Verification items for the finished model (mm, model axes). A direction names the side the tool comes from. Coordinates: 2 decimals unless noted, no trailing zeros. Write each loop counter-clockwise with the first axis right and the second up, starting at its lowest first coordinate (ties: lowest second). Pieces come first, ordered by that corner, then holes. Notation, with made-up numbers: (18.5, -36) -> (27.5, -36) arc R11 ccw to (27.5, -27) -> close; hole circle Ø10 at (73.25, -29.75). An arc over 180 degrees is marked (long way). Answer in a Markdown table with one row per item.
```python
from build123d import *

# Parameters (mm, degrees)
BARREL_PROFILE_SKETCH_R  = 115
BARREL_BODY_230_DEPTH    = 1100
EYE_PIN_HOLE_SKETCH_R    = 50.25
EYE_PIN_HOLE_100_5_DEPTH = 1100
EYE_FLATS_SKETCH_W       = 230
EYE_FLATS_SKETCH_H       = 365
EYE_FLATS_CUT_DEPTH      = 2200
EYE_START                = -117
EYE_BOSS_SKETCH_R        = 115
EYE_BOSS_SKETCH_R_2      = 50.25
EYE_BOSS_EXTRUDE_DEPTH   = 117
EDGE_FILLET_R10_R        = 10


with BuildPart() as part:
    # Barrel Profile Sketch → Barrel Body Ø230 (new, symmetric)
    with BuildSketch(Plane.XY):
        Circle(BARREL_PROFILE_SKETCH_R)
    extrude(amount=BARREL_BODY_230_DEPTH, both=True)

    # Eye Pin Hole Sketch → Eye Pin Hole Ø100.5 (cut, symmetric)
    with BuildSketch(Plane(origin=(0, 0, 0), x_dir=(1, 0, 0), z_dir=(0, 1, 0))):
        with Locations(Location((0, 955, 0), (0, 0, 270))):
            Circle(EYE_PIN_HOLE_SKETCH_R)
    extrude(amount=EYE_PIN_HOLE_100_5_DEPTH, both=True, mode=Mode.SUBTRACT)

    # Eye Flats Sketch → Eye Flats Cut (cut)
    with BuildSketch(Plane(origin=(0, 0, 0), x_dir=(1, 0, 0), z_dir=(0, 1, 0))):
        with Locations((0, 917.5)):
            Rectangle(EYE_FLATS_SKETCH_W, EYE_FLATS_SKETCH_H)
    extrude(amount=-EYE_FLATS_CUT_DEPTH, mode=Mode.SUBTRACT)

    # Eye Transition Sketch → Eye Transition Revolve Cut (revolve, cut)
    with BuildSketch(Plane.XZ):
        with BuildLine():
            Line((-115, -955), (-196.346531204, -955))
            Line((-196.346531204, -955), (-196.346531204, -1191.859792513))
            Line((-196.346531204, -1191.859792513), (0, -1191.859792513))
            Line((0, -1191.859792513), (0, -1070))
            ThreePointArc((0, -1070), (-81.317279836, -1036.317279836), (-115, -955))
        make_face()
    revolve(axis=Axis((0, 0, -1191.859792513), (0, 0, 1)), mode=Mode.SUBTRACT)

    # End Bore Sketch → End Bore Revolve Cut (revolve, cut)
    with BuildSketch(Plane(origin=(0, 0, 0), x_dir=(1, 0, 0), z_dir=(0, 1, 0))):
        Polygon((0, -1100), (61, -1100), (61, -1055.102870795), (81, -1055.102870795), (81, 685), (0, 685), align=None)
    revolve(axis=Axis((0, 0, 1100), (0, 0, -1)), mode=Mode.SUBTRACT)

    # Eye Boss Sketch → Eye Boss Extrude (add)
    with BuildSketch(Plane.XZ.offset(EYE_START)):
        with Locations(Location((0, -955, 0), (0, 0, 270))):
            Circle(EYE_BOSS_SKETCH_R)
        with Locations(Location((0, -955, 0), (0, 0, 90))):
            Circle(EYE_BOSS_SKETCH_R_2, mode=Mode.SUBTRACT)
    extrude(amount=EYE_BOSS_EXTRUDE_DEPTH)

    # Edge Fillet R10
    edge_fillet_r10_edges = [part.edges().sort_by_distance(p)[0] for p in [
        (-115, 0, 1100),
    ]]
    fillet(edge_fillet_r10_edges, radius=EDGE_FILLET_R10_R)


solid = part.part
```
1. Thickness scan on line 1 (Z direction, x = 0, y = 74); line 2 (X direction, y = 0, z = 629); line 3 (Z direction, x = 0, y = 106). Record the ranges inside material, lowest first. Write a range as from..to.
Geometry says:
| item | result |
|---|---|
| line 1 | -1070..-1005.25, -904.75..-685, 1055.1..1100 |
| line 2 | -115..-81, 81..115 |
| line 3 | -1070..-1005.25, -904.75..1099.95 |
2. Mould release check, pull along Z, two halves, no side actions. Record for faces 6 (the cylindrical face through (34.54, 59.32, -1064.69)), 7 (the cylindrical face through (-48.408, 37.118, 1077.237)), 8 (the cylindrical face through (43.545, -68.3, 172.871)): released by +Z, released by -Z, zero draft, split by the parting line, or undercut.
Geometry says:
| item | result |
|---|---|
| face 6 | split by the parting line |
| face 7 | zero draft |
| face 8 | undercut |
3. Section check C-C, the plane z = -796.5. Record the boundary of the cut face in (x, y).
Geometry says:
| item | result |
|---|---|
| outline | (-115, 0) -> (115, 0) arc R115 ccw to start |
4. Depth check by flat-ended pin: P1, Ø2, axis at x = -46, z = 268, coming from the -Y side; P2, Ø1, axis at y = -55.5, z = 714, coming from the -X side; P3, Ø12, axis at y = 1, z = -398.5, coming from the -X side; P4, Ø3, axis at y = -9, z = 705.5, coming from the -X side. Enter the tip coordinate at first touch or a pass-through.
Geometry says:
| item | result |
|---|---|
| P1 | y = -105.83 |
| P2 | x = -101 |
| P3 | x = -115 |
| P4 | x = -114.76 |
5. Section check A-A, the plane x = 0. Record the boundary of the cut face in (y, z), plus the area to 3 significant figures.
Geometry says:
| item | result |
|---|---|
| outline | (-115, -735) -> (0, -735) -> (0, -904.75) -> (117, -904.75) -> (117, -840) -> (115, -840) -> (115, 1090) arc R10 ccw to (105, 1100) -> (61, 1100) -> (61, 1055.1) -> (81, 1055.1) -> (81, -685) -> (-81, -685) -> (-81, 1055.1) -> (-61, 1055.1) -> (-61, 1100) -> (-105, 1100) arc R10 ccw to (-115, 1090) -> close; (0, -1070) -> (117, -1070) -> (117, -1005.25) -> (0, -1005.25) -> close |
| area | 162,000 mm^2 |
6. Section check B-B, the plane z = -503.5. Record the boundary of the cut face in (x, y), plus the area to 3 significant figures.
Geometry says:
| item | result |
|---|---|
| outline | circle Ø230 at (0, 0); hole circle Ø162 at (0, 0) |
| area | 20,900 mm^2 |
7. Tool access check on faces 1 (the cylindrical face through (-14.97, 114.02, 81.81)), 2 (the flat face through (-12, -60, 1055.103)), 3 (the flat face through (-2, -44, -735)), 4 (the flat face through (-50, 117, -979)), 5 (the flat face through (45, -45, 1100)). Record the directions out of +Z, -Z, +X, -X, +Y, -Y that give a thin tool (end or side, any length) a straight path to the whole face; none if there is none.
Geometry says:
| item | result |
|---|---|
| face 1 | +Z |
| face 2 | none |
| face 3 | -Z, +X, -X, -Y |
| face 4 | +Z, -Z, +X, -X, +Y |
| face 5 | +Z, +X, -X, +Y, -Y |
